Geometry check sheet. Reference: the model listing, model coordinates, mm. Round coordinates to 2 decimals unless told otherwise and drop trailing zeros. Order: outer loops, then holes, each group sorted by start corner. A loop starts at its lowest first (then second) coordinate and runs counter-clockwise, first axis right, second up.
(1) Cross-section at C-C on x = 0. Enter the section's corners in (y, z).
(2) Cross-section at A-A on y = -12. Enter the section's corners in (x, z), and give its area (3 significant figures).
(3) Draft check along Y on faces 1 (the face through (11, -12, 2)), 2 (the face through (-8, 0, 0)), 3 (the face through (0, 15, 2)). Enter one of: pulls with the +Y half, pulls with the -Y half, needs draft (parallel to the pull), parting line crosses it, or undercut.
(4) Thickness scan on L1, parallel to Y at x = 12, z = 2.35; L2, parallel to X at y = 3, z = 0.5; L3, parallel to Y at x = 11.25, z = 2.2. Record the ranges inside material, lowest first.
(5) Cross-section at B-B on y = 1.75. Enter the section's corners in (x, z).
from build123d import *

# Parameters (mm, degrees)
SKETCH1_W           = 30
SKETCH1_H           = 30
BOSS_EXTRUDE1_DEPTH = 3
SKETCH2_R           = 1
CUT_EXTRUDE1_DEPTH  = 19
CUT_EXTRUDE2_DEPTH  = 42


with BuildPart() as part:
    # Sketch1 → Boss-Extrude1 (new body)
    with BuildSketch(Plane.XY):
        Rectangle(SKETCH1_W, SKETCH1_H)
    extrude(amount=BOSS_EXTRUDE1_DEPTH)

    # Sketch2 → Cut-Extrude1 (cut)
    with BuildSketch(Plane.XY.offset(3)):
        with Locations((-12, 12)):
            Circle(SKETCH2_R)
        with Locations((12, 12)):
            Circle(SKETCH2_R)
        with Locations((12, -12)):
            Circle(SKETCH2_R)
        with Locations((-12, -12)):
            Circle(SKETCH2_R)
    extrude(amount=-CUT_EXTRUDE1_DEPTH, mode=Mode.SUBTRACT)

    # Sketch3 → Cut-Extrude2 (cut)
    with BuildSketch(Plane.XZ.offset(15)):
        with BuildLine():
            Line((0.95, 0.5), (0.95, 0))
            Line((0.95, 0), (-0.95, 0))
            Line((-0.95, 0), (-0.95, 0.5))
            ThreePointArc((-0.95, 0.5), (0, 1.45), (0.95, 0.5))
        make_face()
    extrude(amount=-CUT_EXTRUDE2_DEPTH, mode=Mode.SUBTRACT)


solid = part.part
Found:
1. outline: (-15, 1.45) - (15, 1.45) - (15, 3) - (-15, 3) - close
2. outline: (-15, 0) - (-13, 0) - (-13, 3) - (-15, 3) - close; (-11, 0) - (-0.95, 0) - (-0.95, 0.5) arc R0.95 cw to (0.95, 0.5) - (0.95, 0) - (11, 0) - (11, 3) - (-11, 3) - close; (13, 0) - (15, 0) - (15, 3) - (13, 3) - close
2. area: 75.6 mm2
3. face 1: undercut
3. face 2: needs draft
3. face 3: pulls with the +Y half
4. L1: y = -15 to -13, -11 to 11, 13 to 15
4. L2: x = -15 to -0.95, 0.95 to 15
4. L3: y = -15 to -12.66, -11.34 to 11.34, 12.66 to 15
5. outline: (-15, 0) - (-0.95, 0) - (-0.95, 0.5) arc R0.95 cw to (0.95, 0.5) - (0.95, 0) - (15, 0) - (15, 3) - (-15, 3) - close
